Source: three-view drawing plus pictorial views. Frame: mm from the lowest corner of the part. A direction names the side the tool comes from. Give positions to 0.01 mm unless a question says otherwise; leave off trailing zeros. Loops run counter-clockwise (first coordinate to the right, second up) from the corner with the lowest first, then second, coordinate; pieces in that order, holes last. Notation, with made-up numbers: (79, -31) - (124, -31) arc R15 cw to (124, -18) - close; hole circle Ø10 at (-36.75, 63.5). An arc over 180 degrees is marked (long way). Write each question's results on one line, items separated by ' | '. Start each with the question number.
(1) Material intervals for line 1 along Y through (x, z) = (8.5, 8.5); line 2 along Y through (x, z) = (3.75, 11.5); line 3 along Z through (x, y) = (8.5, 5) (1 decimal), sorted ascending. Write a range as [from, to].
(2) Reachability of the marked faces 4, 5 and 6 from +Z, -Z, +X, -X, +Y, -Y: full face, straight path, thin tool, end or side. Return the list, or none.
(3) Contact query for flat-ended pins moving along their axis: pin 1 (1.5 mm diameter, centred on x = 7, y = 3.5, fed in from +Z); pin 2 (4 mm diameter, centred on x = 5.5, z = 5, fed in from -Y); pin 3 (2.5 mm diameter, centred on x = 7.5, z = 8, fed in from +Y); pin 4 (1 mm diameter, centred on x = 3, y = 8.5, fed in from -Z). Output: stop coordinate, or through.
(4) Pull-direction query (X, two-part tool) for the marked faces 1, 2 and 3; classes: pulls with the +X half, pulls with the -X half, needs draft (parallel to the pull), parting line crosses it, or undercut.
(5) Cut plane B-B on y = 2.75. Return the cut outline in (x, z).
(6) Cut plane A-A on x = 7. Return the cut outline in (y, z).
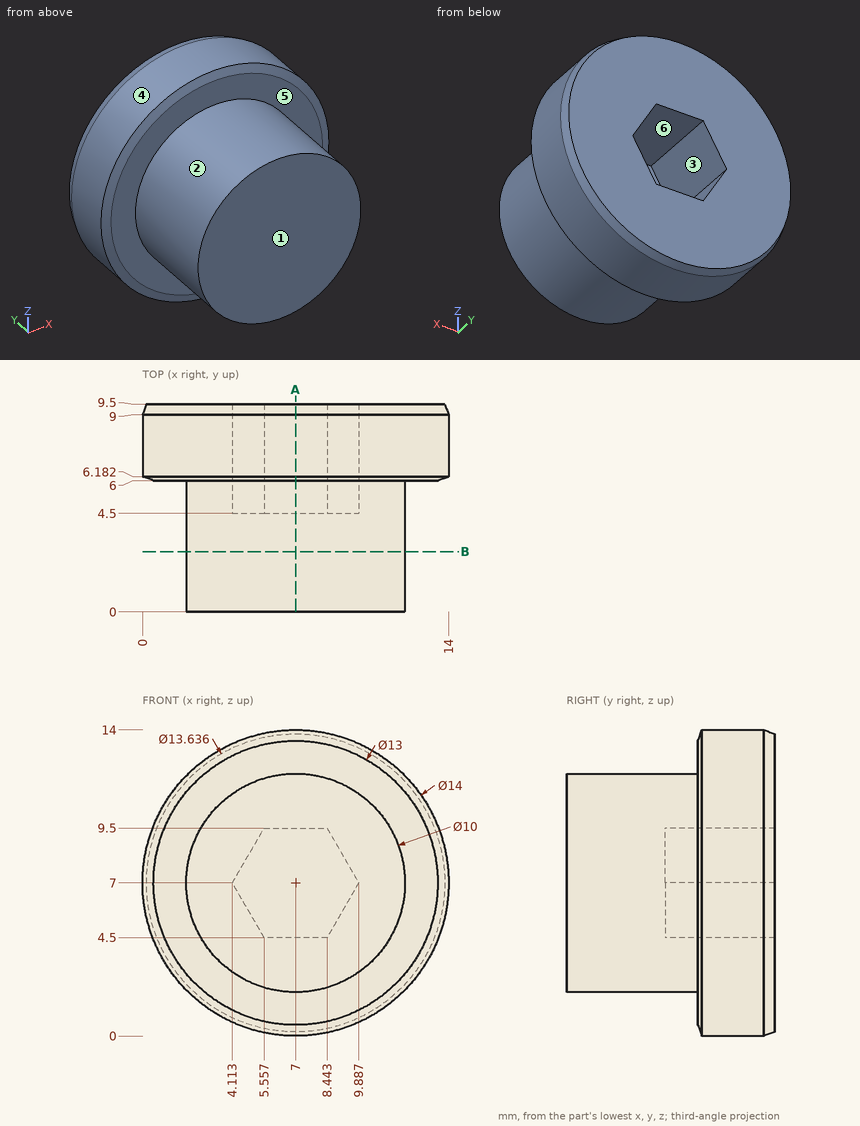
Ans:
1) line 1: [0, 4.5] | line 2: [6, 9.5] | line 3: [2.2, 4.6], [9.4, 11.8]
2) face 4: +Y, -Y | face 5: -Y | face 6: +Y
3) pin 1: z = 12 | pin 2: y = 0 | pin 3: y = 4.5 | pin 4: z = 0.94
4) face 1: needs draft | face 2: parting line crosses it | face 3: undercut
5) outline: circle Ø10 at (7, 7)
6) outline: (0, 2) - (6, 2) - (6, 0.5) - (6.18, 0) - (9, 0) - (9.5, 0.18) - (9.5, 4.5) - (4.5, 4.5) - (4.5, 9.5) - (9.5, 9.5) - (9.5, 13.82) - (9, 14) - (6.18, 14) - (6, 13.5) - (6, 12) - (0, 12) - close
